```python
from build123d import *

# Parameters (mm, degrees)
SKETCH_1_W          = 50
SKETCH_1_H          = 150
EXTRUDE_1_DEPTH     = 5
CUT_EXTRUDE_1_REACH = 81.687
SKETCH_2_R          = 12.75


with BuildPart() as part:
    # 草图1 → 凸台-拉伸1 (new, symmetric)
    with BuildSketch(Plane.XY):
        Rectangle(SKETCH_1_W, SKETCH_1_H)
    extrude(amount=EXTRUDE_1_DEPTH, both=True)

    # 草图2 → 切除-拉伸1 (cut, up to next)
    with BuildSketch(Plane.XY.offset(5), mode=Mode.PRIVATE) as cut_extrude_1_sk1:
        with Locations((0, 45)):
            Circle(SKETCH_2_R)
    cut_extrude_1_tool1 = extrude(cut_extrude_1_sk1.sketch, amount=-CUT_EXTRUDE_1_REACH, mode=Mode.PRIVATE) & part.part
    add(cut_extrude_1_tool1.solids().sort_by_distance((0, 45, 5))[0], mode=Mode.SUBTRACT)


solid = part.part
```
Can you work these out from the model? Positions are in its coordinate system, mm. Coordinates: 2 decimals unless noted, no trailing zeros. Write each loop counter-clockwise with the first axis right and the second up, starting at its lowest first coordinate (ties: lowest second). Pieces come first, ordered by that corner, then holes. Notation, with made-up numbers: M 78,-27.75 L 84,-27.75 A21 cw 84,9.25 Z; hole C 63.5,68 d8. An arc over 180 degrees is marked long. Answer as CSV lines item,"result".
Item 1: We'd pull the mould along X, two halves only. Please class faces 1 (the flat face through (25, -1, 0)), 2 (the cylindrical face through (-2.764, 32.553, 0.07)), 3 (the flat face through (0, -75, 0)), 4 (the flat face through (-25, -1, 0)): +X half, -X half, draft (parallel to the pull), parting line (faces both ways), or undercut.
Geometry results:
face 1,"+X half"
face 2,"undercut"
face 3,"draft"
face 4,"-X half"
Item 2: Imagine slicing it at C-C on z = -1.25. List the corners of the cut face in (x, y) for me, plus the area to 3 significant figures.
Geometry results:
outline,"M -25,-75 L 25,-75 L 25,75 L -25,75 Z; hole C 0,45 d25.5"
area,"6,990 mm2"
Item 3: Please list where these lines run through material, in increasing order: line 1 along Y through (x, z) = (0, -2.25); line 2 along Y through (x, z) = (7, -3).
Geometry results:
line 1,"y = -75 to 32.25, 57.75 to 75"
line 2,"y = -75 to 34.34, 55.66 to 75"
Item 4: Imagine slicing it at A-A on y = 45. List the corners of the cut face in (x, z) for me, plus the area to 3 significant figures.
Geometry results:
outline,"M -25,-5 L -12.75,-5 L -12.75,5 L -25,5 Z; M 12.75,-5 L 25,-5 L 25,5 L 12.75,5 Z"
area,"245 mm2"
Item 5: Imagine slicing it at B-B on x = 0. List the corners of the cut face in (y, z) for me, plus the area to 4 significant figures.
Geometry results:
outline,"M -75,-5 L 32.25,-5 L 32.25,5 L -75,5 Z; M 57.75,-5 L 75,-5 L 75,5 L 57.75,5 Z"
area,"1,245 mm2"
